Could you check a few things on this model? Use its own coordinates, in mm. A direction names the side the tool comes from. Round coordinates to 2 decimals unless told otherwise and drop trailing zeros. Loops run counter-clockwise (first coordinate to the right, second up) from the corner with the lowest first, then second, coordinate; pieces in that order, holes last. Notation, with made-up numbers: (8, 86.5) -> (54, 86.5) arc R25 ccw to (54, 105.5) -> close; hole circle Ø1 at (63.5, 62.5). An arc over 180 degrees is marked (long way). One line per item, written item: value.
```python
from build123d import *

# Parameters (mm, degrees)
SKETCH_1_W                   = 39
SKETCH_1_H                   = 33
EXTRUDE_1_DEPTH              = 10
SKETCH_2_W                   = 39
SKETCH_2_H                   = 10
EXTRUDE_2_DEPTH              = 25
HOLE_WIZARD_M4_1_D           = 3.3
HOLE_WIZARD_M4_1_DEPTH       = 13.5
HOLE_WIZARD_M4_1_TIP         = 0.991420021
HOLE_WIZARD_M5_1_D           = 5.5
HOLE_WIZARD_M5_1_CBORE_D     = 10
HOLE_WIZARD_M5_1_CBORE_DEPTH = 5.4
CHAMFER_1_SIZE               = 0.3


with BuildPart() as part:
    # 草图1 → 凸台-拉伸1 (new body)
    with BuildSketch(Plane(origin=(0, 0, 0), x_dir=(1, 0, 0), z_dir=(0, 1, 0))):
        Rectangle(SKETCH_1_W, SKETCH_1_H)
    extrude(amount=EXTRUDE_1_DEPTH)

    # 草图2 → 凸台-拉伸2 (add)
    with BuildSketch(Plane.XZ):
        with Locations((0, 11.5)):
            Rectangle(SKETCH_2_W, SKETCH_2_H)
    extrude(amount=EXTRUDE_2_DEPTH)

    # M4 螺纹孔1
    with Locations(Plane(origin=(0, 10, 0), x_dir=(1, 0, 0), z_dir=(0, 1, 0))):
        with Locations((11, 11.5), (11, -11.5)):
            Hole(HOLE_WIZARD_M4_1_D / 2, depth=HOLE_WIZARD_M4_1_DEPTH)
            with Locations((0, 0, -(HOLE_WIZARD_M4_1_DEPTH + HOLE_WIZARD_M4_1_TIP / 2))):  # 118° drill point
                Cone(0, HOLE_WIZARD_M4_1_D / 2, HOLE_WIZARD_M4_1_TIP, mode=Mode.SUBTRACT)

    # M5 六角凹头螺钉的柱形沉头孔1 (through all)
    with Locations(Plane(origin=(0, 0, 6.5), x_dir=(-1, 0, 0), z_dir=(0, 0, -1))):
        with Locations((0, -6), (0, -19)):
            CounterBoreHole(HOLE_WIZARD_M5_1_D / 2, HOLE_WIZARD_M5_1_CBORE_D / 2, HOLE_WIZARD_M5_1_CBORE_DEPTH)

    # 倒角1
    chamfer_1_edges = [part.edges().sort_by_distance(p)[0] for p in [
        (0, -25, 16.5),
        (0, -25, 6.5),
        (0, 10, -16.5),
        (0, 0, -16.5),
        (-19.5, 5, -16.5),
        (-19.5, 10, 0),
        (-19.5, 0, -5),
        (-19.5, -12.5, 6.5),
        (-19.5, -25, 11.5),
        (-19.5, -7.5, 16.5),
        (19.5, 10, 0),
        (19.5, 5, -16.5),
        (19.5, 0, -5),
        (19.5, -12.5, 6.5),
        (19.5, -25, 11.5),
        (19.5, -7.5, 16.5),
        (0, 10, 16.5),
    ]]
    chamfer(chamfer_1_edges, length=CHAMFER_1_SIZE)


solid = part.part
```
(1) Please list where these lines run through material, in increasing order: L1, parallel to Z at x = 11, y = 2; L2, parallel to X at y = 2, z = 11.5; L3, parallel to Y at x = 0, z = 10.
Results below:
L1: z = -16.5 to -13.15, -9.85 to 9.85, 13.15 to 16.5
L2: x = -19.5 to 9.35, 12.65 to 19.5
L3: y = -25 to -24, -14 to -11, -1 to 10
(2) Imagine slicing it at A-A on y = -6. Write out the boundary of the cut face in (x, z).
Results below:
outline: (-19.5, 6.8) -> (-19.2, 6.5) -> (-5, 6.5) -> (-5, 11.9) -> (-2.75, 11.9) -> (-2.75, 16.5) -> (-19.2, 16.5) -> (-19.5, 16.2) -> close; (2.75, 11.9) -> (5, 11.9) -> (5, 6.5) -> (19.2, 6.5) -> (19.5, 6.8) -> (19.5, 16.2) -> (19.2, 16.5) -> (2.75, 16.5) -> close
(3) For pin 1 Ø4.5 at (x, y) = (0, -19) entering from +Z; pin 2 Ø12.5 at (x, y) = (-4.5, -10) entering from -Z; pin 3 Ø3 at (x, y) = (0.5, -17.5) entering from -Z, each with a flat end and sliding along its axis, tell me the tip position at first contact or that it passes through.
Results below:
pin 1: passes through
pin 2: stops at z = 6.5
pin 3: stops at z = 11.9
(4) Imagine slicing it at B-B on z = 8. Write out the boundary of the cut face in (x, y), then the cut area to 3 significant figures.
Results below:
outline: (-19.5, -24.7) -> (-19.2, -25) -> (19.2, -25) -> (19.5, -24.7) -> (19.5, 9.7) -> (19.2, 10) -> (-19.2, 10) -> (-19.5, 9.7) -> close; hole circle Ø10 at (0, -19); hole circle Ø10 at (0, -6)
area: 1,210 mm²
(5) Imagine slicing it at C-C on x = 15. Write out the boundary of the cut face in (y, z).
Results below:
outline: (-25, 6.8) -> (-24.7, 6.5) -> (0, 6.5) -> (0, -16.2) -> (0.3, -16.5) -> (9.7, -16.5) -> (10, -16.2) -> (10, 16.2) -> (9.7, 16.5) -> (-24.7, 16.5) -> (-25, 16.2) -> close
(6) Imagine slicing it at D-D on y = -13.5. Write out the boundary of the cut face in (x, z).
Results below:
outline: (-19.5, 6.8) -> (-19.2, 6.5) -> (19.2, 6.5) -> (19.5, 6.8) -> (19.5, 16.2) -> (19.2, 16.5) -> (-19.2, 16.5) -> (-19.5, 16.2) -> close
(7) On a 3-axis mill with a long thin cutter (end or side, diameter ignored), from which of +Z, -Z, +X, -X, +Y, -Y can I reach the whole of each face in a straight line? I mean faces 5 (the face through (-2.2, -8.2, 11.9)), 6 (the face through (9.476, 3.156, 12.132)), 7 (the face through (0, -12, 6.5)). Say none if no direction works.
Results below:
face 5: -Z
face 6: +Y
face 7: -Z, +X, -X, -Y
(8) We'd pull the mould along Z, two halves only. Please class faces 1 (the face through (-19.5, -3, 7)), 2 (the face through (0, -11, 16.5)), 3 (the face through (-2.2, -21.2, 11.9)), 4 (the face through (10.239, 4.93, -10.036)): +Z half, -Z half, draft (parallel to the pull), parting line (faces both ways), or undercut.
Results below:
face 1: draft
face 2: +Z half
face 3: -Z half
face 4: undercut
